```python
from build123d import *

# Parameters (mm, degrees)
SKETCH1_R           = 16
SKETCH1_R_2         = 2
BOSS_EXTRUDE1_DEPTH = 60
SKETCH2_W           = 5
SKETCH2_H           = 0.1
BOSS_EXTRUDE2_DEPTH = 20
SKETCH3_W           = 5
SKETCH3_H           = 0.1
BOSS_EXTRUDE3_DEPTH = 20


with BuildPart() as part:
    # Sketch1 → Boss-Extrude1 (new body)
    with BuildSketch(Plane.XY):
        Circle(SKETCH1_R)
        Circle(SKETCH1_R_2, mode=Mode.SUBTRACT)
    extrude(amount=BOSS_EXTRUDE1_DEPTH)

    # Sketch2 → Boss-Extrude2 (add)
    with BuildSketch(Plane(origin=(0, 0, 0), x_dir=(-1, 0, 0), z_dir=(0, 0, -1))):
        with Locations((0, 5.05)):
            Rectangle(SKETCH2_W, SKETCH2_H)
    extrude(amount=BOSS_EXTRUDE2_DEPTH)

    # Sketch3 → Boss-Extrude3 (add)
    with BuildSketch(Plane.XY.offset(60)):
        with Locations((0, 8.05)):
            Rectangle(SKETCH3_W, SKETCH3_H)
        with Locations((0, 2.55)):
            Rectangle(SKETCH3_W, SKETCH3_H)
    extrude(amount=BOSS_EXTRUDE3_DEPTH)


solid = part.part
```
Geometry: final body of the model. Coordinates: model frame, mm. Coordinates: 2 decimals unless noted, no trailing zeros. Write each loop counter-clockwise with the first axis right and the second up, starting at its lowest first coordinate (ties: lowest second). Pieces come first, ordered by that corner, then holes. Notation, with made-up numbers: M -32.75,63.5 L -25.75,63.5 A34 cw -25.75,100.5 Z; hole C -1.75,33 d11. An arc over 180 degrees is marked long. Use CSV: the item, a comma, the result in double quotes. Start each with the question number.
1. Cut plane C-C on z = 10. Return the cut outline in (x, y).
2. Cut plane B-B on x = 0. Return the cut outline in (y, z), plus the area to 3 significant figures.
3. First-contact query: P1, Ø5.5, axis at x = 1, z = 66.5, coming from the +Y side; P2, Ø5, axis at y = -10, z = 54.5, coming from the +X side; P3, Ø8, axis at x = 3.5, z = 6.5, coming from the +Y side; P4, Ø2, axis at x = -9, y = -11, coming from the -Z side. Flat tips, straight axial feed; report the tip coordinate or a pass-through.
4. Ray query, probe 1 along Y at (x, z) = (0, 41.5); probe 2 along Z at (x, y) = (-9, -1); probe 3 along Y at (x, z) = (1.5, 31.5). Return the intervals inside material, ascending.
5. Cut plane A-A on y = 0. Return the cut outline in (x, z).
6. Cut plane D-D on z = -12.5. Return the cut outline in (x, y), plus the area to 3 significant figures.
7. Mould query, pull axis Y, two halves, no side actions, for faces 1 (the face through (-3.47, -15.62, 29.58)), 2 (the face through (3, 0, 0)), 3 (the face through (0, -2, 30)). Classes: pulls with the +Y half, pulls with the -Y half, needs draft (parallel to the pull), parting line crosses it, or undercut.
Entries:
1,outline,"C 0,0 d32; hole C 0,0 d4"
2,outline,"M -16,0 L -2,0 L -2,60 L -16,60 Z; M 2,0 L 5,0 L 5,-20 L 5.1,-20 L 5.1,0 L 16,0 L 16,60 L 8.1,60 L 8.1,80 L 8,80 L 8,60 L 2.6,60 L 2.6,80 L 2.5,80 L 2.5,60 L 2,60 Z"
2,area,"1,690 mm²"
3,P1,"y = 8.1"
3,P2,"x = 14.13"
3,P3,"y = 16"
3,P4,"z = 0"
4,probe 1,"-16 to -2, 2 to 16"
4,probe 2,"0 to 60"
4,probe 3,"-15.93 to -1.32, 1.32 to 15.93"
5,outline,"M -16,0 L -2,0 L -2,60 L -16,60 Z; M 2,0 L 16,0 L 16,60 L 2,60 Z"
6,outline,"M -2.5,5 L 2.5,5 L 2.5,5.1 L -2.5,5.1 Z"
6,area,"0.500 mm²"
7,face 1,"parting line crosses it"
7,face 2,"needs draft"
7,face 3,"undercut"
